Check sheet for the modelled part. Datum: model origin and axes. Units: mm. A direction names the side the tool comes from. Give positions to 0.01 mm unless a question says otherwise; leave off trailing zeros. Order: outer loops, then holes, each group sorted by start corner. A loop starts at its lowest first (then second) coordinate and runs counter-clockwise, first axis right, second up. Notation, with made-up numbers: (21.25, 22) -> (79.25, 22) arc R15 ccw to (79.25, 38) -> close; hole circle Ø4 at (-32.5, -25.5). An arc over 180 degrees is marked (long way). Write each question's results on one line, items separated by ' | '.
from build123d import *

# Parameters (mm, degrees)
SKETCH1_W            = 120
SKETCH1_H            = 100
BOSS_EXTRUDE1_DEPTH  = 5
CUT_EXTRUDE1_DEPTH   = 157.284996081
MIRROR2_COPY_1_DEPTH = 157.284996081
BOSS_EXTRUDE2_DEPTH  = 250
CUT_EXTRUDE2_DEPTH   = 450


with BuildPart() as part:
    # Sketch1 → Boss-Extrude1 (new body)
    with BuildSketch(Plane(origin=(0, 0, 0), x_dir=(1, 0, 0), z_dir=(0, 1, 0))):
        with Locations((60, 50)):
            Rectangle(SKETCH1_W, SKETCH1_H)
    extrude(amount=BOSS_EXTRUDE1_DEPTH)

    # Sketch2 → Cut-Extrude1 (cut, through all)
    with BuildSketch(Plane(origin=(0, 5, 0), x_dir=(1, 0, 0), z_dir=(0, 1, 0))):
        with BuildLine():
            Line((13.012661712, 92.320396367), (13.012661712, 82.342416735))
            ThreePointArc((13.012661712, 82.342416735), (8.883842554, 78.213597578), (4.755023397, 82.342416735))
            Line((4.755023397, 82.342416735), (4.755023397, 92.320396367))
            ThreePointArc((4.755023397, 92.320396367), (8.883842554, 96.449215524), (13.012661712, 92.320396367))
        make_face()
    cut_extrude1 = extrude(amount=-CUT_EXTRUDE1_DEPTH, mode=Mode.SUBTRACT)

    # Mirror1: Cut-Extrude1 across plane
    add(cut_extrude1.mirror(Plane.ZY.offset(-60)), mode=Mode.SUBTRACT)

    # Mirror2: Cut-Extrude1 across plane
    add(cut_extrude1.mirror(Plane.XY.offset(-50)), mode=Mode.SUBTRACT)

    # Mirror2 copy 1 sketch → Mirror2 copy 1 (cut, through all)
    with BuildSketch(Plane(origin=(120, 5, -100), x_dir=(-1, 0, 0), z_dir=(0, 1, 0))):
        with BuildLine():
            Line((13.012661712, 92.320396367), (13.012661712, 82.342416735))
            ThreePointArc((13.012661712, 82.342416735), (8.883842554, 78.213597578), (4.755023397, 82.342416735))
            Line((4.755023397, 82.342416735), (4.755023397, 92.320396367))
            ThreePointArc((4.755023397, 92.320396367), (8.883842554, 96.449215524), (13.012661712, 92.320396367))
        make_face()
    extrude(amount=-MIRROR2_COPY_1_DEPTH, mode=Mode.SUBTRACT)

    # Sketch4 → Boss-Extrude2 (add)
    with BuildSketch(Plane.XZ):
        Polygon((2.5, -50), (2.5, -75), (7.5, -75), (7.5, -50), (7.5, -25), (2.5, -25), align=None)
        Polygon((112.5, -75), (117.5, -75), (117.5, -45), (117.5, -25), (112.5, -25), (112.5, -45), align=None)
    extrude(amount=BOSS_EXTRUDE2_DEPTH)

    # Sketch5 → Cut-Extrude2 (cut)
    with BuildSketch(Plane.ZY.offset(-2.5)):
        with BuildLine():
            Line((-60.5, -250), (-60.5, -220))
            ThreePointArc((-60.5, -220), (-50, -209.5), (-39.5, -220))
            Line((-39.5, -220), (-39.5, -250))
            ThreePointArc((-39.5, -250), (-50, -260.5), (-60.5, -250))
        make_face()
    extrude(amount=-CUT_EXTRUDE2_DEPTH, mode=Mode.SUBTRACT)


solid = part.part
1. Section check B-B on z = -71. Record the cut outline in (x, y).
Verdict:
outline: (0, 0) -> (2.5, 0) -> (2.5, -250) -> (7.5, -250) -> (7.5, 0) -> (112.5, 0) -> (112.5, -250) -> (117.5, -250) -> (117.5, 0) -> (120, 0) -> (120, 5) -> (0, 5) -> close
2. Section check D-D on z = -50. Record the cut outline in (x, y), then the cut area to 4 significant figures.
Verdict:
outline: (0, 0) -> (2.5, 0) -> (2.5, -209.5) -> (7.5, -209.5) -> (7.5, 0) -> (112.5, 0) -> (112.5, -209.5) -> (117.5, -209.5) -> (117.5, 0) -> (120, 0) -> (120, 5) -> (0, 5) -> close | area: 2,695 mm^2
3. Mould release check, pull along Z, two halves, no side actions. Record for faces 6 (the flat face through (115, -123, -25)), 7 (the cylindrical face through (5, -209.5, -50.2)), 8 (the flat face through (112.5, -123, -50)): +Z half, -Z half, draft (parallel to the pull), parting line (faces both ways), or undercut.
Verdict:
face 6: +Z half | face 7: undercut | face 8: draft
4. Gauge pin test, flat ends, axial feed: pin 1 Ø5.5 at (x, y) = (115, -232.5) entering from +Z; pin 2 Ø5.5 at (x, y) = (4.5, -96.5) entering from -Z; pin 3 Ø15 at (y, z) = (-154, -38) entering from -X. Record the tip position at first contact, or that the pin passes through.
Verdict:
pin 1: stops at z = -25 | pin 2: stops at z = -75 | pin 3: stops at x = 2.5
5. Section check A-A on y = -167. Record the cut outline in (x, z).
Verdict:
outline: (2.5, -75) -> (7.5, -75) -> (7.5, -25) -> (2.5, -25) -> close; (112.5, -75) -> (117.5, -75) -> (117.5, -25) -> (112.5, -25) -> close
6. Material ranges on probe 1 along X at (y, z) = (-67, -65); probe 2 along Y at (x, z) = (48, -11.5), recorded low to high. Write a range as from..to.
Verdict:
probe 1: x = 2.5..7.5, 112.5..117.5 | probe 2: y = 0..5
7. Section check C-C on x = 84.5. Record the cut outline in (y, z).
Verdict:
outline: (0, -100) -> (5, -100) -> (5, 0) -> (0, 0) -> close
8. Access from +Z, -Z, +X, -X, +Y, -Y to the whole of each face (thin tool, end or side, straight path). Record for faces 1 (the flat face through (5, -235, -39.5)), 2 (the flat face through (5, -250, -68)), 3 (the flat face through (13.013, 3, -87)), 4 (the flat face through (115, -123, -75)), 5 (the flat face through (7.5, -123, -50)).
Verdict:
face 1: +X, -X, -Y | face 2: +Z, -Z, +X, -X, -Y | face 3: +Y, -Y | face 4: -Z, +X, -X, -Y | face 5: +Z, -Z, -Y
